```python
from build123d import *

# Parameters (mm, degrees)
SKETCH_1_W                   = 55
SKETCH_1_H                   = 40
EXTRUDE_1_DEPTH              = 8
SKETCH_2_W                   = 35
SKETCH_2_H                   = 16
CUT_EXTRUDE_1_DEPTH          = 35.932076949
HOLE_WIZARD_M3_1_D           = 3.4
HOLE_WIZARD_M3_1_CBORE_D     = 6
HOLE_WIZARD_M3_1_CBORE_DEPTH = 3.4
HOLE_WIZARD_M3_1_2_D         = 2.5
HOLE_WIZARD_M3_1_2_DEPTH     = 7.5
HOLE_WIZARD_M3_1_2_TIP       = 0.751075774
M8X1_0_1_D                   = 5
M8X1_0_1_CBORE_D             = 8
M8X1_0_1_CBORE_DEPTH         = 6
HOLE_WIZARD_M3_2_D           = 2.5
HOLE_WIZARD_M3_2_DEPTH       = 8.5
HOLE_WIZARD_M3_2_TIP         = 0.751075774
CHAMFER_1_SIZE               = 3
FILLET_1_R                   = 5


with BuildPart() as part:
    # 草图1 → 凸台-拉伸1 (new body)
    with BuildSketch(Plane.XY.offset(4)):
        Rectangle(SKETCH_1_W, SKETCH_1_H)
    extrude(amount=-EXTRUDE_1_DEPTH)

    # 草图2 → 切除-拉伸1 (cut, through all)
    with BuildSketch(Plane(origin=(0, 0, -4), x_dir=(-1, 0, 0), z_dir=(0, 0, -1))):
        Rectangle(SKETCH_2_W, SKETCH_2_H)
    extrude(amount=-CUT_EXTRUDE_1_DEPTH, mode=Mode.SUBTRACT)

    # Hole Wizard M3 _1 (through all)
    with Locations(Plane(origin=(0, 0, -4), x_dir=(-1, 0, 0), z_dir=(0, 0, -1))):
        with Locations((10, -12.5), (-10, -12.5), (10, 12.5), (-10, 12.5)):
            CounterBoreHole(HOLE_WIZARD_M3_1_D / 2, HOLE_WIZARD_M3_1_CBORE_D / 2, HOLE_WIZARD_M3_1_CBORE_DEPTH)

    # Hole Wizard M3 _1 2
    with Locations(Plane(origin=(27.5, 0, 0), x_dir=(0, 0, -1), z_dir=(1, 0, 0))):
        with Locations((0, 6), (0, -6)):
            Hole(HOLE_WIZARD_M3_1_2_D / 2, depth=HOLE_WIZARD_M3_1_2_DEPTH)
            with Locations((0, 0, -(HOLE_WIZARD_M3_1_2_DEPTH + HOLE_WIZARD_M3_1_2_TIP / 2))):  # 118° drill point
                Cone(0, HOLE_WIZARD_M3_1_2_D / 2, HOLE_WIZARD_M3_1_2_TIP, mode=Mode.SUBTRACT)

    # M8x1.0 螺纹孔1 (through all)
    with Locations(Plane.XY.offset(4)):
        with Locations((-20, 12.5), (-20, -12.5), (20, 12.5), (20, -12.5)):
            CounterBoreHole(M8X1_0_1_D / 2, M8X1_0_1_CBORE_D / 2, M8X1_0_1_CBORE_DEPTH)

    # M3 螺纹孔2
    with Locations(Plane.ZY.offset(27.5)):
        with Locations((0, 6), (0, -6)):
            Hole(HOLE_WIZARD_M3_2_D / 2, depth=HOLE_WIZARD_M3_2_DEPTH)
            with Locations((0, 0, -(HOLE_WIZARD_M3_2_DEPTH + HOLE_WIZARD_M3_2_TIP / 2))):  # 118° drill point
                Cone(0, HOLE_WIZARD_M3_2_D / 2, HOLE_WIZARD_M3_2_TIP, mode=Mode.SUBTRACT)

    # 倒角1
    chamfer_1_edges = [part.edges().sort_by_distance(p)[0] for p in [
        (27.5, 20, 0),
        (27.5, -20, 0),
        (-27.5, -20, 0),
        (-27.5, 20, 0),
    ]]
    chamfer(chamfer_1_edges, length=CHAMFER_1_SIZE)

    # 圆角1
    fillet_1_edges = [part.edges().sort_by_distance(p)[0] for p in [
        (-17.5, -8, 0),
        (17.5, -8, 0),
        (17.5, 8, 0),
        (-17.5, 8, 0),
    ]]
    fillet(fillet_1_edges, radius=FILLET_1_R)


solid = part.part
```
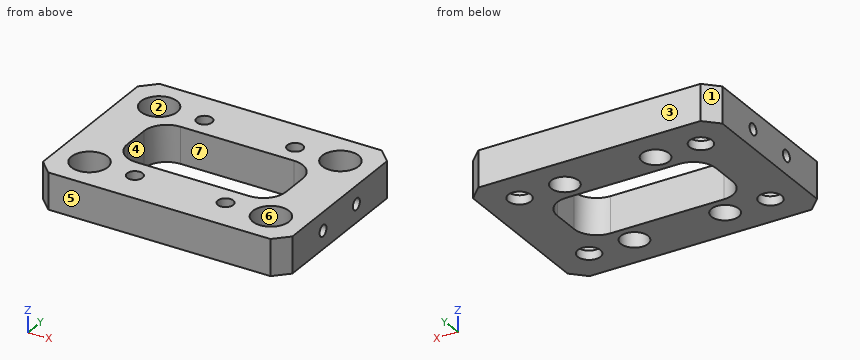
Could you check a few things on this model? Use its own coordinates, in mm. Face numbers are marked on the shaded views. A direction names the side the tool comes from. Round coordinates to 2 decimals unless told otherwise and drop trailing zeros. Loops run counter-clockwise (first coordinate to the right, second up) from the corner with the lowest first, then second, coordinate; pieces in that order, holes last. Notation, with made-up numbers: (70.25, 50) -> (91.25, 50) arc R28 cw to (91.25, 79) -> close; hole circle Ø9 at (-6.75, -15). An arc over 180 degrees is marked (long way). Put each result on its own line as item: value.
Q1. Thinking about a two-plate mould opening in X: for the marked faces 1, 2, 3 and 4, which applies, pulls with the +X half, pulls with the -X half, needs draft (parallel to the pull), parting line crosses it, or undercut?
Checks:
face 1: pulls with the -X half
face 2: undercut
face 3: needs draft
face 4: undercut
Q2. I want a section at B-B on z = 2.25. Give the number of separate pieces and of enclosed holes in the cut face, and give its area (3 significant figures).
Checks:
separate pieces: 1
enclosed holes: 9
area: 1,410 mm2
Q3. I want a section at C-C on x = -4.5. Write out the boundary of the cut face in (y, z), and give its area (3 significant figures).
Checks:
outline: (-20, -4) -> (-8, -4) -> (-8, 4) -> (-20, 4) -> close; (8, -4) -> (20, -4) -> (20, 4) -> (8, 4) -> close
area: 192 mm2
Q4. Which directions (+Z, -Z, +X, -X, +Y, -Y) give clear straight access to the entire face, cutting with the end or side of a thin tool? Please do the marked faces 5, 6 and 7.
Checks:
face 5: +Z, -Z, +X, -X, -Y
face 6: +Z
face 7: +Z, -Z
Q5. Please list where these lines run through material, in increasing order: line 1 (Y direction, x = 20, z = 2.7); line 2 (Y direction, x = -10, z = -1.95); line 3 (Y direction, x = -20, z = -2.65). Write a range as from..to.
Checks:
line 1: -20..-16.5, -8.5..8.5, 16.5..20
line 2: -20..-15.5, -9.5..-8, 8..9.5, 15.5..20
line 3: -20..-15, -10..10, 15..20
Q6. For pin 1 Ø5.5 at (x, y) = (10, 12.5) entering from -Z, with a flat end and sliding along its axis, tell me the tip position at first contact or that it passes through.
Checks:
pin 1: z = -0.6
Q7. I want a section at D-D on x = -10. Write out the boundary of the cut face in (y, z), and give its area (3 significant figures).
Checks:
outline: (-20, -4) -> (-15.5, -4) -> (-15.5, -0.6) -> (-14.2, -0.6) -> (-14.2, 4) -> (-20, 4) -> close; (-10.8, -0.6) -> (-9.5, -0.6) -> (-9.5, -4) -> (-8, -4) -> (-8, 4) -> (-10.8, 4) -> close; (8, -4) -> (9.5, -4) -> (9.5, -0.6) -> (10.8, -0.6) -> (10.8, 4) -> (8, 4) -> close; (14.2, -0.6) -> (15.5, -0.6) -> (15.5, -4) -> (20, -4) -> (20, 4) -> (14.2, 4) -> close
area: 120 mm2
Q8. I want a section at A-A on x = -20. Write out the boundary of the cut face in (y, z), and give its area (3 significant figures).
Checks:
outline: (-20, -4) -> (-15, -4) -> (-15, -2) -> (-16.5, -2) -> (-16.5, 4) -> (-20, 4) -> close; (-10, -4) -> (10, -4) -> (10, -2) -> (8.5, -2) -> (8.5, 4) -> (-8.5, 4) -> (-8.5, -2) -> (-10, -2) -> close; (15, -4) -> (20, -4) -> (20, 4) -> (16.5, 4) -> (16.5, -2) -> (15, -2) -> close; hole circle Ø2.5 at (-6, 0); hole circle Ø2.5 at (6, 0)
area: 194 mm2
